```python
from build123d import *

# Parameters (mm, degrees)
SKETCH1_W                                           = 45
SKETCH1_H                                           = 50
BOSS_EXTRUDE1_DEPTH                                 = 12
CBORE_FOR_M8_HEX_SOCKET_HEAD_CAP_SCREW1_D           = 9
CBORE_FOR_M8_HEX_SOCKET_HEAD_CAP_SCREW1_CBORE_D     = 15
CBORE_FOR_M8_HEX_SOCKET_HEAD_CAP_SCREW1_CBORE_DEPTH = 8.6
CHAMFER1_SIZE                                       = 2


with BuildPart() as part:
    # Sketch1 → Boss-Extrude1 (new body)
    with BuildSketch(Plane.XY):
        Rectangle(SKETCH1_W, SKETCH1_H)
    extrude(amount=BOSS_EXTRUDE1_DEPTH)

    # CBORE for M8 Hex Socket Head Cap Screw1 (through all)
    with Locations(Plane.XY.offset(12)):
        with Locations((-12, 16), (12, 16), (12, -16), (-12, -16)):
            CounterBoreHole(CBORE_FOR_M8_HEX_SOCKET_HEAD_CAP_SCREW1_D / 2, CBORE_FOR_M8_HEX_SOCKET_HEAD_CAP_SCREW1_CBORE_D / 2, CBORE_FOR_M8_HEX_SOCKET_HEAD_CAP_SCREW1_CBORE_DEPTH)

    # Chamfer1
    chamfer1_edges = [part.edges().sort_by_distance(p)[0] for p in [
        (22.5, -25, 6),
        (-22.5, -25, 6),
        (-22.5, 25, 6),
        (22.5, 25, 6),
    ]]
    chamfer(chamfer1_edges, length=CHAMFER1_SIZE)


solid = part.part
```
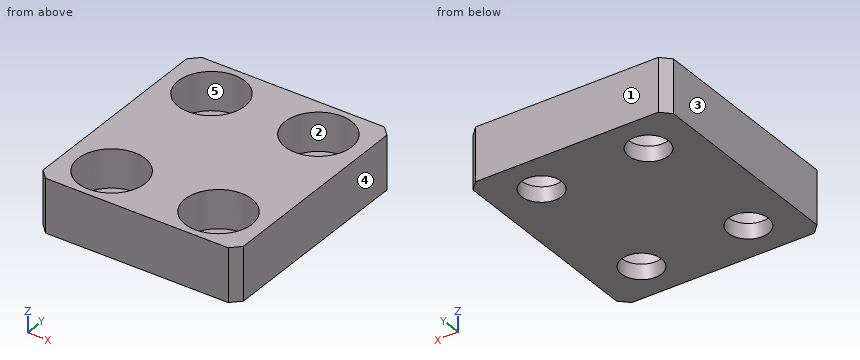
For this review, take the finished solid that the model builds, in its own axes (mm). Face numbers are marked on the shaded views. A direction names the side the tool comes from. Coordinates: 2 decimals unless noted, no trailing zeros. Write each loop counter-clockwise with the first axis right and the second up, starting at its lowest first coordinate (ties: lowest second). Pieces come first, ordered by that corner, then holes.
(1) Add section D-D on x = 6. Give the boundary of the cut face in (y, z).
(2) Wall thickness on probe 1 along Y at (x, z) = (-12, 2.25); probe 2 along Y at (x, z) = (-12, 7.25); probe 3 along X at (y, z) = (13, 2): over which ranges is each line inside the solid? List them lowest first.
(3) Add section C-C on z = 8.5. Give the boundary of the cut face in (x, y).
(4) The part is to be moulded in two halves that separate along X. For the marked faces 3, 4 and 5, say which applies: +X half, -X half, draft (parallel to the pull), parting line (faces both ways), or undercut.
(5) Tool access review of the marked faces 1 and 2: name each direction out of +Z, -Z, +X, -X, +Y, -Y from which nothing blocks a thin tool from reaching the whole face with its end or side.
(6) Add section B-B on x = -12. Give the boundary of the cut face in (y, z).
(7) Add section A-A on y = -16. Give the boundary of the cut face in (x, z), then the cut area to 3 significant figures.
(8) For pin 1 Ø7 at (x, y) = (12, -16) entering from -Z; pin 2 Ø11.5 at (x, y) = (-12, 16) entering from +Z, all flat-tipped, find the tip position at first contact; note any pin that passes through.
Answer sheet:
1. outline: (-25, 0) - (25, 0) - (25, 12) - (20.5, 12) - (20.5, 3.4) - (11.5, 3.4) - (11.5, 12) - (-11.5, 12) - (-11.5, 3.4) - (-20.5, 3.4) - (-20.5, 12) - (-25, 12) - close
2. probe 1: y = -25 to -20.5, -11.5 to 11.5, 20.5 to 25
2. probe 2: y = -25 to -23.5, -8.5 to 8.5, 23.5 to 25
2. probe 3: x = -22.5 to -15.35, -8.65 to 8.65, 15.35 to 22.5
3. outline: (-22.5, -23) - (-20.5, -25) - (20.5, -25) - (22.5, -23) - (22.5, 23) - (20.5, 25) - (-20.5, 25) - (-22.5, 23) - close; hole circle Ø15 at (-12, -16); hole circle Ø15 at (-12, 16); hole circle Ø15 at (12, -16); hole circle Ø15 at (12, 16)
4. face 3: -X half
4. face 4: +X half
4. face 5: undercut
5. face 1: +Z, -Z, +X, -X, +Y
5. face 2: +Z
6. outline: (-25, 0) - (-20.5, 0) - (-20.5, 3.4) - (-23.5, 3.4) - (-23.5, 12) - (-25, 12) - close; (-11.5, 0) - (11.5, 0) - (11.5, 3.4) - (8.5, 3.4) - (8.5, 12) - (-8.5, 12) - (-8.5, 3.4) - (-11.5, 3.4) - close; (20.5, 0) - (25, 0) - (25, 12) - (23.5, 12) - (23.5, 3.4) - (20.5, 3.4) - close
7. outline: (-22.5, 0) - (-16.5, 0) - (-16.5, 3.4) - (-19.5, 3.4) - (-19.5, 12) - (-22.5, 12) - close; (-7.5, 0) - (7.5, 0) - (7.5, 3.4) - (4.5, 3.4) - (4.5, 12) - (-4.5, 12) - (-4.5, 3.4) - (-7.5, 3.4) - close; (16.5, 0) - (22.5, 0) - (22.5, 12) - (19.5, 12) - (19.5, 3.4) - (16.5, 3.4) - close
7. area: 221 mm2
8. pin 1: passes through
8. pin 2: stops at z = 3.4
